from build123d import *

# Parameters (mm, degrees)
SKETCH1_R           = 4
BOSS_EXTRUDE1_DEPTH = 20
BOSS_EXTRUDE2_DEPTH = 6


with BuildPart() as part:
    # Sketch1 → Boss-Extrude1 (new body)
    with BuildSketch(Plane.XY):
        Circle(SKETCH1_R)
    extrude(amount=BOSS_EXTRUDE1_DEPTH)

    # Sketch2 → Boss-Extrude2 (add)
    with BuildSketch(Plane.XY.offset(20)):
        Polygon((-3.75, 6.495190528), (-7.5, 0), (-3.75, -6.495190528), (3.75, -6.495190528), (7.5, 0), (3.75, 6.495190528), align=None)
    extrude(amount=BOSS_EXTRUDE2_DEPTH)


solid = part.part
Input: part model. Units: mm. Frame: model coordinates. A direction names the side the tool comes from. Round coordinates to 2 decimals unless told otherwise and drop trailing zeros. Order: outer loops, then holes, each group sorted by start corner. A loop starts at its lowest first (then second) coordinate and runs counter-clockwise, first axis right, second up.
1. Cut plane A-A, the plane x = 0. Output: boundary loops of the cut face in (y, z), then the cut area to 3 significant figures.
The answers:
outline: (-6.5, 20) - (-4, 20) - (-4, 0) - (4, 0) - (4, 20) - (6.5, 20) - (6.5, 26) - (-6.5, 26) - close
area: 238 mm2
2. Cut plane C-C, the plane z = 16.25. Output: boundary loops of the cut face in (x, y).
The answers:
outline: circle Ø8 at (0, 0)
3. Cut plane D-D, the plane x = -6.25. Output: boundary loops of the cut face in (y, z), then the cut area to 3 significant figures.
The answers:
outline: (-2.17, 20) - (2.17, 20) - (2.17, 26) - (-2.17, 26) - close
area: 26.0 mm2
4. Set-up query: faces 1 (the face through (0, 6.495, 23)), 2 (the face through (-0.867, -3.905, 9.86)). Return all of +Z, -Z, +X, -X, +Y, -Y with unobstructed straight access to the full face (end or side cutting, diameter ignored); none if empty.
The answers:
face 1: +Z, -Z, +X, -X, +Y
face 2: -Z
5. Material intervals for line 1 (Z direction, x = 3.5, y = 4.25); line 2 (Y direction, x = 0, z = 11.75); line 3 (Y direction, x = 3.25, z = 13.75), sorted ascending.
The answers:
line 1: z = 20 to 26
line 2: y = -4 to 4
line 3: y = -2.33 to 2.33
6. Cut plane B-B, the plane y = -1. Output: boundary loops of the cut face in (x, z), then the cut area to 3 significant figures.
The answers:
outline: (-6.92, 20) - (-3.87, 20) - (-3.87, 0) - (3.87, 0) - (3.87, 20) - (6.92, 20) - (6.92, 26) - (-6.92, 26) - close
area: 238 mm2
7. Pin query (flat end, axial travel): P1, Ø1, axis at y = 4, z = 8, coming from the -X side; P2, Ø3, axis at x = 1, z = 11, coming from the -Y side; P3, Ø1.5, axis at y = -1, z = 13, coming from the +X side. Return the tip coordinate at first contact, or that it passes through.
The answers:
P1: stops at x = -1.94
P2: stops at y = -4
P3: stops at x = 3.99
